from build123d import *

# Parameters (mm, degrees)
SKETCH1_W                  = 55
SKETCH1_H                  = 18
BOSS_EXTRUDE1_DEPTH        = 30
SKETCH2_R                  = 4
CUT_EXTRUDE1_DEPTH         = 25
SKETCH3_R                  = 2.5
CUT_EXTRUDE2_DEPTH         = 38
SKETCH4_W                  = 75
SKETCH4_H                  = 27
SKETCH4_R                  = 4
BOSS_EXTRUDE2_DEPTH        = 10
BOSS_EXTRUDE3_START        = 10
SKETCH6_W                  = 75
SKETCH6_H                  = 18
SKETCH6_R                  = 4
BOSS_EXTRUDE3_DEPTH        = 10
SKETCH7_W                  = 75
SKETCH7_H                  = 20
CUT_EXTRUDE3_DEPTH         = 31
SKETCH8_R                  = 1.280962141
CUT_EXTRUDE4_DEPTH         = 24
F_8_2_8_2_DIAMETER_HOLE1_D = 8
CHAMFER1_SIZE              = 2
SKETCH10_R                 = 2.5
CUT_EXTRUDE5_DEPTH         = 25
SKETCH11_R                 = 1.362041629
CUT_EXTRUDE6_DEPTH         = 10
M4_TAPPED_HOLE1_D          = 3.3
M4_TAPPED_HOLE1_DEPTH      = 10.1
M4_TAPPED_HOLE1_TIP        = 0.991420021
SKETCH13_W                 = 55
SKETCH13_H                 = 5
CUT_EXTRUDE7_DEPTH         = 22
CHAMFER2_SIZE              = 0.5
CHAMFER3_SIZE              = 1


with BuildPart() as part:
    # Sketch1 → Boss-Extrude1 (new body)
    with BuildSketch(Plane(origin=(0, 0, 0), x_dir=(1, 0, 0), z_dir=(0, 1, 0))):
        Rectangle(SKETCH1_W, SKETCH1_H)
    extrude(amount=BOSS_EXTRUDE1_DEPTH)

    # Sketch2 → Cut-Extrude1 (cut)
    with BuildSketch(Plane(origin=(0, 30, 0), x_dir=(1, 0, 0), z_dir=(0, 1, 0))):
        with Locations(Location((-20, 0, 0), (0, 0, 270))):
            Circle(SKETCH2_R)
        with Locations(Location((20, 0, 0), (0, 0, 90))):
            Circle(SKETCH2_R)
    extrude(amount=-CUT_EXTRUDE1_DEPTH, mode=Mode.SUBTRACT)

    # Sketch3 → Cut-Extrude2 (cut)
    with BuildSketch(Plane(origin=(0, 30, 0), x_dir=(1, 0, 0), z_dir=(0, 1, 0))):
        with Locations(Location((-20, 0, 0), (0, 0, 270))):
            Circle(SKETCH3_R)
        with Locations(Location((20, 0, 0), (0, 0, 270))):
            Circle(SKETCH3_R)
    extrude(amount=-CUT_EXTRUDE2_DEPTH, mode=Mode.SUBTRACT)

    # Sketch4 → Boss-Extrude2 (add)
    with BuildSketch(Plane(origin=(0, 30, 0), x_dir=(1, 0, 0), z_dir=(0, 1, 0))):
        Rectangle(SKETCH4_W, SKETCH4_H)
        with Locations(Location((-20, 0, 0), (0, 0, 270))):
            Circle(SKETCH4_R, mode=Mode.SUBTRACT)
        with Locations(Location((20, 0, 0), (0, 0, 90))):
            Circle(SKETCH4_R, mode=Mode.SUBTRACT)
    extrude(amount=-BOSS_EXTRUDE2_DEPTH)

    # Sketch6 → Boss-Extrude3 (add)
    with BuildSketch(Plane(origin=(0, 30, 0), x_dir=(1, 0, 0), z_dir=(0, 1, 0)).offset(BOSS_EXTRUDE3_START)):
        Rectangle(SKETCH6_W, SKETCH6_H)
        with Locations(Location((-20, 0, 0), (0, 0, 270))):
            Circle(SKETCH6_R, mode=Mode.SUBTRACT)
        with Locations(Location((20, 0, 0), (0, 0, 270))):
            Circle(SKETCH6_R, mode=Mode.SUBTRACT)
    extrude(amount=-BOSS_EXTRUDE3_DEPTH)

    # Sketch7 → Cut-Extrude3 (cut)
    with BuildSketch(Plane.XY.offset(13.5)):
        with Locations((0, 30)):
            Rectangle(SKETCH7_W, SKETCH7_H)
    extrude(amount=-CUT_EXTRUDE3_DEPTH, mode=Mode.SUBTRACT)

    # Sketch8 → Cut-Extrude4 (cut)
    with BuildSketch(Plane(origin=(0, 20, 0), x_dir=(1, 0, 0), z_dir=(0, 1, 0))):
        with Locations(Location((0, 0, 0), (0, 0, 270))):
            Circle(SKETCH8_R)
    extrude(amount=-CUT_EXTRUDE4_DEPTH, mode=Mode.SUBTRACT)

    # Ø8.2 (8.2) Diameter Hole1 (through all)
    with Locations(Plane.ZX.offset(20)):
        with Locations((0, 0)):
            Hole(F_8_2_8_2_DIAMETER_HOLE1_D / 2)

    # Chamfer1
    chamfer1_edges = [part.edges().sort_by_distance(p)[0] for p in [
        (-27.5, 0, 0),
        (27.5, 0, 0),
    ]]
    chamfer(chamfer1_edges, length=CHAMFER1_SIZE)

    # Sketch10 → Cut-Extrude5 (cut)
    with BuildSketch(Plane(origin=(0, 20, 0), x_dir=(1, 0, 0), z_dir=(0, 1, 0))):
        with Locations(Location((-10, 0, 0), (0, 0, 270))):
            Circle(SKETCH10_R)
        with Locations(Location((10, 0, 0), (0, 0, 270))):
            Circle(SKETCH10_R)
    extrude(amount=-CUT_EXTRUDE5_DEPTH, mode=Mode.SUBTRACT)

    # Sketch11 → Cut-Extrude6 (cut)
    with BuildSketch(Plane.XY.offset(9)):
        with Locations((0, 8)):
            Circle(SKETCH11_R)
    extrude(amount=-CUT_EXTRUDE6_DEPTH, mode=Mode.SUBTRACT)

    # M4 Tapped Hole1
    with Locations(Plane(origin=(0, 8, 9), x_dir=(1, 0, 0), z_dir=(0, 0, 1))):
        with Locations((0, 0)):
            Hole(M4_TAPPED_HOLE1_D / 2, depth=M4_TAPPED_HOLE1_DEPTH)
            with Locations((0, 0, -(M4_TAPPED_HOLE1_DEPTH + M4_TAPPED_HOLE1_TIP / 2))):  # 118° drill point
                Cone(0, M4_TAPPED_HOLE1_D / 2, M4_TAPPED_HOLE1_TIP, mode=Mode.SUBTRACT)

    # Sketch13 → Cut-Extrude7 (cut)
    with BuildSketch(Plane.XY.offset(9)):
        with Locations((0, 17.5)):
            Rectangle(SKETCH13_W, SKETCH13_H)
    extrude(amount=-CUT_EXTRUDE7_DEPTH, mode=Mode.SUBTRACT)

    # Chamfer2
    chamfer2_edges = [part.edges().sort_by_distance(p)[0] for p in [
        (-10, 0, -2.5),
        (10, 0, -2.5),
        (10, 15, -2.5),
        (-10, 15, -2.5),
    ]]
    chamfer(chamfer2_edges, length=CHAMFER2_SIZE)

    # Chamfer3
    chamfer3_edges = [part.edges().sort_by_distance(p)[0] for p in [
        (-20, 15, -4),
        (20, 15, 4),
    ]]
    chamfer(chamfer3_edges, length=CHAMFER3_SIZE)


solid = part.part
Input: part model. Units: mm. Frame: model coordinates. A direction names the side the tool comes from. Coordinates: 2 decimals unless noted, no trailing zeros. Loops run counter-clockwise (first coordinate to the right, second up) from the corner with the lowest first, then second, coordinate; pieces in that order, holes last.
(1) Section A-A on x = 10. Return the cut outline in (y, z).
(2) Section C-C on x = 0. Return the cut outline in (y, z), then the cut area to 4 significant figures.
(3) Section D-D on z = 6. Return the cut outline in (x, y), then the cut area to 3 significant figures.
(4) Pull-direction query (Z, two-part tool) for faces 1 (the face through (-18, 5, 2)), 2 (the face through (7.56, 7.6, -0.54)), 3 (the face through (0, 6, 9)), 4 (the face through (27.5, 8, 0)); classes: released by +Z, released by -Z, zero draft, split by the parting line, or undercut.
(5) Material intervals for probe 1 along X at (y, z) = (7, 0); probe 2 along X at (y, z) = (4.75, 0); probe 3 along Z at (x, y) = (0, 4), sorted ascending.
(6) Set-up query: faces 5 (the face through (0.215, 9.636, 6.284)), 6 (the face through (-12.44, 7.6, -0.54)). Return all of +Z, -Z, +X, -X, +Y, -Y with unobstructed straight access to the full face (end or side cutting, diameter ignored); none if empty.
(7) First-contact query: pin 1 Ø6.5 at (x, z) = (18.5, 0.5) entering from +Y; pin 2 Ø2.5 at (x, y) = (0, 8) entering from +Z; pin 3 Ø6.5 at (x, z) = (20, 0) entering from +Y; pin 4 Ø4.5 at (x, z) = (10, 0) entering from +Y. Flat tips, straight axial feed; report the tip coordinate or a pass-through.
Data:
1. outline: (0, -9) - (15, -9) - (15, -3) - (14.5, -2.5) - (0.5, -2.5) - (0, -3) - close; (0, 3) - (0.5, 2.5) - (14.5, 2.5) - (15, 3) - (15, 9) - (0, 9) - close
2. outline: (0, -9) - (15, -9) - (15, -4) - (0, -4) - close; (0, 4) - (6.35, 4) - (6.35, 9) - (0, 9) - close; (9.65, 4) - (15, 4) - (15, 9) - (9.65, 9) - close
2. area: 133.5 mm2
3. outline: (-27.5, 2) - (-25.5, 0) - (25.5, 0) - (27.5, 2) - (27.5, 15) - (-27.5, 15) - close; hole circle Ø3.3 at (0, 8)
3. area: 812 mm2
4. face 1: undercut
4. face 2: undercut
4. face 3: released by +Z
4. face 4: zero draft
5. probe 1: x = -27.5 to -24, -16 to -12.5, -7.5 to -4, 4 to 7.5, 12.5 to 16, 24 to 27.5
5. probe 2: x = -27.5 to -22.5, -17.5 to -12.5, -7.5 to -4, 4 to 7.5, 12.5 to 17.5, 22.5 to 27.5
5. probe 3: z = -9 to -4, 4 to 9
6. face 5: +Z
6. face 6: +Y, -Y
7. pin 1: stops at y = 14.83
7. pin 2: stops at z = -3.8
7. pin 3: stops at y = 5
7. pin 4: passes through
